Could you check a few things on this model? Use its own coordinates, in mm. Face numbers are marked on the shaded views. Round coordinates to 2 decimals unless told otherwise and drop trailing zeros. Loops run counter-clockwise (first coordinate to the right, second up) from the corner with the lowest first, then second, coordinate; pieces in that order, holes last. Notation, with made-up numbers: (60.25, 88.5) -> (71.25, 88.5) arc R13 cw to (71.25, 98.5) -> close; hole circle Ø4 at (-0.75, -19.5). An arc over 180 degrees is marked (long way). One line per item, written item: value.
```python
from build123d import *

# Parameters (mm, degrees)
SKETCH1_R           = 5
BOSS_EXTRUDE1_DEPTH = 80
CUT_EXTRUDE2_DEPTH  = 3


with BuildPart() as part:
    # Sketch1 → Boss-Extrude1 (new body)
    with BuildSketch(Plane.XY):
        Circle(SKETCH1_R)
    extrude(amount=BOSS_EXTRUDE1_DEPTH)

    # Sketch2 → Cut-Extrude2 (cut)
    with BuildSketch(Plane(origin=(0, 5, 0), x_dir=(1, 0, 0), z_dir=(0, 1, 0))):
        with BuildLine():
            Line((-1.519571935, -15), (-1.519571935, -3.259754454))
            ThreePointArc((-1.519571935, -3.259754454), (0, -1.740182518), (1.519571935, -3.259754454))
            Line((1.519571935, -3.259754454), (1.519571935, -15))
            ThreePointArc((1.519571935, -15), (0, -16.519571935), (-1.519571935, -15))
        make_face()
    extrude(amount=-CUT_EXTRUDE2_DEPTH, mode=Mode.SUBTRACT)


solid = part.part
```
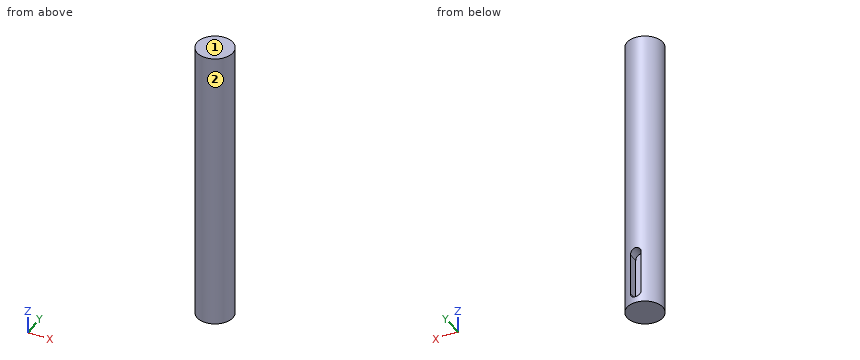
(1) Imagine slicing it at D-D on y = -3.5. Write out the boundary of the cut face in (x, z), then the cut area to 3 significant figures.
Results below:
outline: (-3.57, 0) -> (3.57, 0) -> (3.57, 80) -> (-3.57, 80) -> close
area: 571 mm²
(2) Imagine slicing it at B-B on x = 0. Write out the boundary of the cut face in (y, z).
Results below:
outline: (-5, 0) -> (5, 0) -> (5, 1.74) -> (2, 1.74) -> (2, 16.52) -> (5, 16.52) -> (5, 80) -> (-5, 80) -> close
(3) Imagine slicing it at A-A on y = 4. Write out the boundary of the cut face in (x, z), then the cut area to 3 significant figures.
Results below:
outline: (-3, 0) -> (3, 0) -> (3, 80) -> (-3, 80) -> close; hole (-1.52, 3.26) arc R1.52 ccw to (1.52, 3.26) -> (1.52, 15) arc R1.52 ccw to (-1.52, 15) -> close
area: 437 mm²
(4) For pin 1 Ø2.5 at (x, z) = (-0.5, 9.5) entering from +Y; pin 2 Ø1 at (x, z) = (0, 9) entering from +Y; pin 3 Ø1.5 at (x, z) = (3, 54) entering from +Y, each with a flat end and sliding along its axis, tell me the tip position at first contact or that it passes through.
Results below:
pin 1: stops at y = 4.76
pin 2: stops at y = 2
pin 3: stops at y = 4.47
(5) We'd pull the mould along X, two halves only. Please class the marked faces 1 and 2: +X half, -X half, draft (parallel to the pull), parting line (faces both ways), or undercut.
Results below:
face 1: draft
face 2: parting line
(6) Imagine slicing it at C-C on z = 50.5. Write out the boundary of the cut face in (x, y).
Results below:
outline: circle Ø10 at (0, 0)
(7) Please list where these lines run through material, in increasing order: L1, parallel to X at y = -0.25, z = 67.5; L2, parallel to Z at x = 0.75, y = 4.5; L3, parallel to Y at x = -1.25, z = 55.5.
Results below:
L1: x = -4.99 to 4.99
L2: z = 0 to 1.94, 16.32 to 80
L3: y = -4.84 to 4.84
